Here's how the part is built. I have some questions about the finished solid (model axes, mm). Face numbers are marked on the shaded views. A direction names the side the tool comes from. Coordinates: 2 decimals unless noted, no trailing zeros. Loops run counter-clockwise (first coordinate to the right, second up) from the corner with the lowest first, then second, coordinate; pieces in that order, holes last.
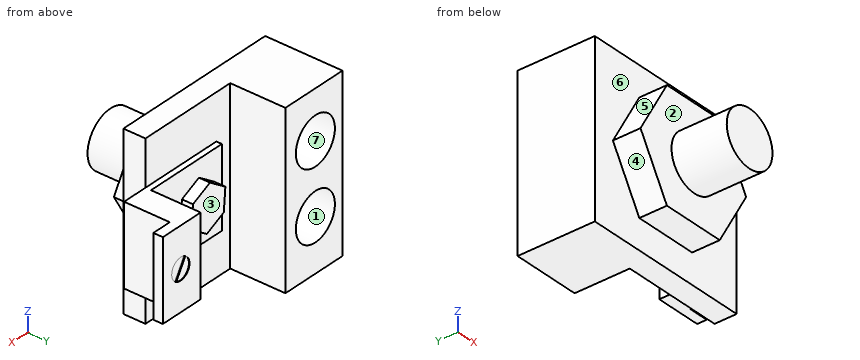
```python
from build123d import *

# Parameters (mm, degrees)
BOSS_EXTRUDE1_DEPTH = 5
SKETCH2_R           = 5
BOSS_EXTRUDE2_DEPTH = 10
SKETCH3_W           = 31.008368254
SKETCH3_H           = 30.751916894
BOSS_EXTRUDE3_DEPTH = 4
SKETCH4_W           = 12.473016313
SKETCH4_H           = 30.751916894
BOSS_EXTRUDE4_DEPTH = 10
SKETCH5_W           = 20.18023145
SKETCH5_H           = 14.400921404
BOSS_EXTRUDE5_DEPTH = 1
BOSS_EXTRUDE6_DEPTH = 14.400921404
SKETCH7_R           = 4.270954595
CUT_EXTRUDE1_DEPTH  = 11
SKETCH8_R           = 1.943003429
CUT_EXTRUDE2_DEPTH  = 0.1
CUT_EXTRUDE3_DEPTH  = 0.1
BOSS_EXTRUDE7_DEPTH = 2


with BuildPart() as part:
    # Sketch1 → Boss-Extrude1 (new body)
    with BuildSketch(Plane(origin=(0, 0, 0), x_dir=(1, 0, 0), z_dir=(0, 1, 0))):
        Polygon((5.773502692, 10), (-5.773502692, 10), (-11.547005384, 0), (-5.773502692, -10), (5.773502692, -10), (11.547005384, 0), align=None)
    extrude(amount=BOSS_EXTRUDE1_DEPTH)

    # Sketch2 → Boss-Extrude2 (add)
    with BuildSketch(Plane.XZ):
        with Locations(Location((0.234789437, 0, 0), (0, 0, 270))):
            Circle(SKETCH2_R)
    extrude(amount=BOSS_EXTRUDE2_DEPTH)

    # Sketch3 → Boss-Extrude3 (add)
    with BuildSketch(Plane(origin=(0, 5, 0), x_dir=(1, 0, 0), z_dir=(0, 1, 0))):
        Rectangle(SKETCH3_W, SKETCH3_H)
    extrude(amount=BOSS_EXTRUDE3_DEPTH)

    # Sketch4 → Boss-Extrude4 (add)
    with BuildSketch(Plane(origin=(0, 9, 0), x_dir=(1, 0, 0), z_dir=(0, 1, 0))):
        with Locations((-9.267675971, 0)):
            Rectangle(SKETCH4_W, SKETCH4_H)
    extrude(amount=BOSS_EXTRUDE4_DEPTH)

    # Sketch5 → Boss-Extrude5 (add)
    with BuildSketch(Plane(origin=(0, 9, 0), x_dir=(1, 0, 0), z_dir=(0, 1, 0))):
        with Locations((10.090115725, 0)):
            Rectangle(SKETCH5_W, SKETCH5_H)
    extrude(amount=BOSS_EXTRUDE5_DEPTH)

    # Sketch6 → Boss-Extrude6 (add)
    with BuildSketch(Plane.XY.offset(7.200460702)):
        Polygon((20.18023145, 10), (20.18023145, 17.284010358), (23.772647306, 17.284010358), (23.772647306, 19), (15.494895542, 19), (15.494895542, 10), align=None)
    extrude(amount=-BOSS_EXTRUDE6_DEPTH)

    # Sketch7 → Cut-Extrude1 (cut)
    with BuildSketch(Plane(origin=(0, 19, 0), x_dir=(1, 0, 0), z_dir=(0, 1, 0))):
        with Locations(Location((-9.583665468, 5.917314438, 0), (0, 0, 270))):
            Circle(SKETCH7_R)
        with Locations(Location((-9.583665468, -6.64552011, 0), (0, 0, 270))):
            Circle(SKETCH7_R)
    extrude(amount=-CUT_EXTRUDE1_DEPTH, mode=Mode.SUBTRACT)

    # Sketch8 → Cut-Extrude2 (cut)
    with BuildSketch(Plane(origin=(0, 19, 0), x_dir=(1, 0, 0), z_dir=(0, 1, 0))):
        with Locations(Location((19.889507686, 0, 0), (0, 0, 270))):
            Circle(SKETCH8_R)
    extrude(amount=-CUT_EXTRUDE2_DEPTH, mode=Mode.SUBTRACT)

    # Sketch9 → Cut-Extrude3 (cut)
    with BuildSketch(Plane(origin=(0, 18.9, 0), x_dir=(1, 0, 0), z_dir=(0, 1, 0))):
        Polygon((18.714185293, -1.560675462), (20.714119659, 1.771187657), (21.064830078, 1.560675462), (19.064895713, -1.771187657), align=None)
    extrude(amount=-CUT_EXTRUDE3_DEPTH, mode=Mode.SUBTRACT)

    # Sketch10 → Boss-Extrude7 (add)
    with BuildSketch(Plane(origin=(0, 10, 0), x_dir=(1, 0, 0), z_dir=(0, 1, 0))):
        Polygon((5.703266191, 4.088977096), (1.990998258, 2.340859575), (1.648778474, -1.748117521), (5.018826623, -4.088977096), (8.731094556, -2.340859575), (9.07331434, 1.748117521), align=None)
    extrude(amount=BOSS_EXTRUDE7_DEPTH)


solid = part.part
```
1. I want a section at B-B (x = 8). Please give me the cut outline in (y, z).
2. We'd pull the mould along Z, two halves only. Please class the marked faces 5, 6 and 7: +Z half, -Z half, draft (parallel to the pull), parting line (faces both ways), or undercut.
3. I want a section at A-A (y = 15.75). Please give me the cut outline in (x, z).
4. I need wall thicknesses on line 1 along Z through (x, y) = (-9.5, 17.5); line 2 along X through (y, z) = (17, 0); line 3 along Y through (x, z) = (22.5, -3). Which ranges of each line are inside material? Lowest first, please.
5. On a 3-axis mill with a long thin cutter (end or side, diameter ignored), from which of +Z, -Z, +X, -X, +Y, -Y can I reach the whole of each face in a straight line? I mean the marked faces 1, 2, 3 and 4. Say none if no direction works.
6. I want a section at D-D (y = 2). Please give me the cut outline in (x, z), then the cut area to 3 significant figures.
7. For pin 1 (10 mm diameter, centred on y = 7, z = -8.5, fed in from +X); pin 2 (2 mm diameter, centred on x = 7, z = -7, fed in from +Y); pin 3 (7 mm diameter, centred on x = -8.5, z = 6.5, fed in from +Y); pin 4 (8 mm diameter, centred on y = -7, z = -3, fed in from -X), each with a flat end and sliding along its axis, tell me the tip position at first contact or that it passes through.
Response values:
1. outline: (0, -6.14) - (5, -6.14) - (5, -15.38) - (9, -15.38) - (9, -7.2) - (10, -7.2) - (10, -2.49) - (12, -2.49) - (12, 2.69) - (10, 2.69) - (10, 7.2) - (9, 7.2) - (9, 15.38) - (5, 15.38) - (5, 6.14) - (0, 6.14) - close
2. face 5: +Z half
2. face 6: draft
2. face 7: undercut
3. outline: (-15.5, -15.38) - (-3.03, -15.38) - (-3.03, 15.38) - (-15.5, 15.38) - close; (15.49, -7.2) - (20.18, -7.2) - (20.18, 7.2) - (15.49, 7.2) - close; hole circle Ø8.54 at (-9.58, -5.92); hole circle Ø8.54 at (-9.58, 6.65)
4. line 1: z = -15.38 to -10.19, -1.65 to 2.38, 10.92 to 15.38
4. line 2: x = -15.5 to -3.03, 15.49 to 20.18
4. line 3: y = 17.28 to 19
5. face 1: +Y
5. face 2: -Y
5. face 3: +Z, -Z, +Y
5. face 4: -Z, -X, -Y
6. outline: (-11.55, 0) - (-5.77, -10) - (5.77, -10) - (11.55, 0) - (5.77, 10) - (-5.77, 10) - close
6. area: 346 mm2
7. pin 1: stops at x = 20.18
7. pin 2: stops at y = 10
7. pin 3: stops at y = 19
7. pin 4: stops at x = -4.77
